```python
from build123d import *

# Parameters (mm, degrees)
BOSS_EXTRUDE1_DEPTH = 20


with BuildPart() as part:
    # Sketch1 → Boss-Extrude1 (new body)
    with BuildSketch(Plane.XY):
        Polygon((9106.725741881, 4668.311117452), (9575.225782872, 4668.311117452), (9575.225782872, 4418.311117452), (9106.725741967, 4418.311117452), align=None)
        with BuildLine():
            Line((9247.225783525, 4568.310529412), (9247.225783525, 4518.311318924))
            ThreePointArc((9247.225783525, 4518.311318924), (9272.225682554, 4493.311117122), (9297.225783432, 4518.311117075))
            Line((9297.225783432, 4518.311117075), (9297.225783432, 4568.311116981))
            ThreePointArc((9297.225783432, 4568.311116981), (9272.225489694, 4593.31082315), (9247.225783525, 4568.310529412))
        make_face(mode=Mode.SUBTRACT)
    extrude(amount=BOSS_EXTRUDE1_DEPTH)


solid = part.part
```
CAD build for the part. Positions are in the model's coordinates, mm. A direction names the side the tool comes from. Give positions to 0.01 mm unless a question says otherwise; leave off trailing zeros. Write each loop counter-clockwise with the first axis right and the second up, starting at its lowest first coordinate (ties: lowest second). Pieces come first, ordered by that corner, then holes. Notation, with made-up numbers: (71, 56.5) -> (93, 56.5) arc R28 ccw to (93, 94.5) -> close; hole circle Ø2 at (-31, 19). An arc over 180 degrees is marked (long way). Write each question's results on one line, items separated by ' | '.
1. Two-plate mould, pull along X, no slides. Class faces 3 (the flat face through (9575.226, 4545, 10)), 4 (the cylindrical face through (9272.775, 4593.305, 9.86)), 5 (the flat face through (9344, 4545, 20)): pulls with the +X half, pulls with the -X half, needs draft (parallel to the pull), parting line crosses it, or undercut.
Geometry check:
face 3: pulls with the +X half | face 4: undercut | face 5: needs draft
2. Which spindle directions (+Z, -Z, +X, -X, +Y, -Y) get a long thin tool onto all of the face, cutting with end or side? Do faces 1 (the flat face through (9344, 4418.311, 10)), 2 (the cylindrical face through (9271.676, 4493.317, 9.86)). Say none if no direction does.
Geometry check:
face 1: +Z, -Z, +X, -X, -Y | face 2: +Z, -Z
3. Cut at C-C, the plane x = 9258.5. Write the cut outline in (y, z).
Geometry check:
outline: (4418.31, 0) -> (4497.42, 0) -> (4497.42, 20) -> (4418.31, 20) -> close; (4589.21, 0) -> (4668.31, 0) -> (4668.31, 20) -> (4589.21, 20) -> close
4. Cut at A-A, the plane y = 4525. Write the cut outline in (x, z).
Geometry check:
outline: (9106.73, 0) -> (9247.23, 0) -> (9247.23, 20) -> (9106.73, 20) -> close; (9297.23, 0) -> (9575.23, 0) -> (9575.23, 20) -> (9297.23, 20) -> close
5. Cut at B-B, the plane z = 3.5. Write the cut outline in (x, y), then the cut area to 3 significant figures.
Geometry check:
outline: (9106.73, 4418.31) -> (9575.23, 4418.31) -> (9575.23, 4668.31) -> (9106.73, 4668.31) -> close; hole (9247.23, 4518.31) arc R25 ccw to (9297.23, 4518.31) -> (9297.23, 4568.31) arc R25 ccw to (9247.23, 4568.31) -> close | area: 113,000 mm²
6. Wall check: probe 1 along X at (y, z) = (4549, 12.25); probe 2 along X at (y, z) = (4508.5, 4); probe 3 along Y at (x, z) = (9262.5, 3). Give the ranges that are in metal, low to high. Write a range as [from, to].
Geometry check:
probe 1: [9106.73, 9247.23], [9297.23, 9575.23] | probe 2: [9106.73, 9249.23], [9295.22, 9575.23] | probe 3: [4418.31, 4495.28], [4591.34, 4668.31]
